Part model, mm, in its own coordinate system. A direction names the side the tool comes from. Give positions to 0.01 mm unless a question says otherwise; leave off trailing zeros. Order: outer loops, then holes, each group sorted by start corner. A loop starts at its lowest first (then second) coordinate and runs counter-clockwise, first axis right, second up. Notation, with made-up numbers: (86.25, 2.5) - (135.25, 2.5) arc R8 cw to (135.25, 17.5) - close; hole circle Ø11 at (57.5, -11.75). An arc over 180 degrees is marked (long way). One line per item, written item: value.
```python
from build123d import *

# Parameters (mm, degrees)
L_BRACKET_BODY_DEPTH          = 47.5
UPRIGHT_ROUND_TOP_DEPTH       = 40
HUB_BOSS_40_SKETCH_R          = 20
HUB_BOSS_40_DEPTH             = 8
BEARING_BORE_30_SKETCH_R      = 15
BEARING_BORE_30_DEPTH         = 65
CLAMP_BORE_40_WITH_SLOT_DEPTH = 65
CLAMP_SCREW_HOLE_10_SKETCH_R  = 5
CLAMP_SCREW_HOLE_10_DEPTH     = 253.833937595


with BuildPart() as part:
    # L-Bracket Profile Sketch → L-Bracket Body (new, symmetric)
    with BuildSketch(Plane.XY):
        with BuildLine():
            Line((0, 0), (150, 0))
            Line((150, 0), (150, 20))
            Line((150, 20), (75, 40))
            Line((75, 40), (55, 40))
            ThreePointArc((55, 40), (44.393398282, 44.393398282), (40, 55))
            Line((40, 55), (40, 132.5))
            Line((40, 132.5), (0, 132.5))
            Line((0, 132.5), (0, 0))
        make_face()
    extrude(amount=L_BRACKET_BODY_DEPTH, both=True)

    # Upright Round Top Sketch → Upright Round Top (add)
    with BuildSketch(Plane.ZY):
        with BuildLine():
            Line((-47.5, 132.5), (47.5, 132.5))
            ThreePointArc((47.5, 132.5), (0, 180), (-47.5, 132.5))
        make_face()
    extrude(amount=-UPRIGHT_ROUND_TOP_DEPTH)

    # Hub Boss Ø40 Sketch → Hub Boss Ø40 (add)
    with BuildSketch(Plane(origin=(40, 0, 0), x_dir=(0, 0, -1), z_dir=(1, 0, 0))):
        with Locations(Location((0, 132.5, 0), (0, 0, 270))):
            Circle(HUB_BOSS_40_SKETCH_R)
    extrude(amount=HUB_BOSS_40_DEPTH)

    # Bearing Bore Ø30 Sketch → Bearing Bore Ø30 (cut)
    with BuildSketch(Plane(origin=(48, 0, 0), x_dir=(0, 0, -1), z_dir=(1, 0, 0))):
        with Locations(Location((0, 132.5, 0), (0, 0, 90))):
            Circle(BEARING_BORE_30_SKETCH_R)
    extrude(amount=-BEARING_BORE_30_DEPTH, mode=Mode.SUBTRACT)

    # Clamp Bore Ø40 Slot Sketch → Clamp Bore Ø40 with Slot (cut)
    with BuildSketch(Plane(origin=(0, 40, 0), x_dir=(1, 0, 0), z_dir=(0, 1, 0))):
        with BuildLine():
            Line((150, 5), (150, -5))
            Line((150, -5), (129.364916731, -5))
            ThreePointArc((129.364916731, -5), (110, -20), (90.635083269, -5))
            Line((90.635083269, -5), (55, -5))
            Line((55, -5), (55, 5))
            Line((55, 5), (90.635083269, 5))
            ThreePointArc((90.635083269, 5), (110, 20), (129.364916731, 5))
            Line((129.364916731, 5), (150, 5))
        make_face()
    extrude(amount=-CLAMP_BORE_40_WITH_SLOT_DEPTH, mode=Mode.SUBTRACT)

    # Clamp Screw Hole Ø10 Sketch → Clamp Screw Hole Ø10 (cut, through all)
    with BuildSketch(Plane.XY.offset(47.5)):
        with Locations((140, 10)):
            Circle(CLAMP_SCREW_HOLE_10_SKETCH_R)
    extrude(amount=-CLAMP_SCREW_HOLE_10_DEPTH, mode=Mode.SUBTRACT)


solid = part.part
```
1) Slice it at C-C on x = 113.5. Write the cut outline in (y, z).
Answer:
outline: (0, -47.5) - (29.73, -47.5) - (29.73, -19.69) - (0, -19.69) - close; (0, 19.69) - (29.73, 19.69) - (29.73, 47.5) - (0, 47.5) - close
2) Slice it at D-D on z = 0. Write the cut outline in (x, y).
Answer:
outline: (0, 0) - (55, 0) - (55, 40) arc R15 cw to (40, 55) - (40, 112.5) - (48, 112.5) - (48, 117.5) - (0, 117.5) - close; (0, 147.5) - (48, 147.5) - (48, 152.5) - (40, 152.5) - (40, 180) - (0, 180) - close
3) Drop flat-ended pins along their axis: P1, Ø12, axis at x = 32.5, z = -3.5, coming from the +Y side; P2, Ø22, axis at x = 67.5, z = -17.5, coming from the +Y side; P3, Ø12, axis at x = 89.5, z = 31.5, coming from the +Y side. Give the stop position or say it passes through.
Answer:
P1: stops at y = 180
P2: stops at y = 40
P3: stops at y = 37.73
4) Slice it at B-B on y = 10. Write the cut outline in (x, z).
Answer:
outline: (0, -47.5) - (135, -47.5) - (135, -5) - (129.36, -5) arc R20 cw to (90.64, -5) - (55, -5) - (55, 5) - (90.64, 5) arc R20 cw to (129.36, 5) - (135, 5) - (135, 47.5) - (0, 47.5) - close; (145, -47.5) - (150, -47.5) - (150, -5) - (145, -5) - close; (145, 5) - (150, 5) - (150, 47.5) - (145, 47.5) - close
5) Slice it at A-A on z = 11. Write the cut outline in (x, y).
Answer:
outline: (0, 0) - (93.3, 0) - (93.3, 35.12) - (75, 40) - (55, 40) arc R15 cw to (40, 55) - (40, 115.8) - (48, 115.8) - (48, 122.3) - (0, 122.3) - close; (0, 142.7) - (48, 142.7) - (48, 149.2) - (40, 149.2) - (40, 178.71) - (0, 178.71) - close; (126.7, 0) - (150, 0) - (150, 20) - (126.7, 26.21) - close; hole circle Ø10 at (140, 10)
6) Which spindle directions (+Z, -Z, +X, -X, +Y, -Y) get a long thin tool onto all of the face, cutting with end or side? Do faces 1 (the face through (65, 40, -26)), 2 (the face through (40, 104, -1)), 3 (the face through (140, 16, 5)), 4 (the face through (110, 14, 20)). Say none if no direction does.
Answer:
face 1: +Z, -Z, +X, +Y
face 2: +X
face 3: +X, +Y, -Y
face 4: +Y, -Y
7) Wall check: line 1 along Z through (x, y) = (30.5, 132.5); line 2 along X through (y, z) = (124, 20). Give the ranges that are in metal, low to high. Write a range as [from, to].
Answer:
line 1: z = [-47.5, -15], [15, 47.5]
line 2: x = [0, 40]
8) Two-plate mould, pull along Z, no slides. Class faces 5 (the face through (55, 20, 0)), 6 (the face through (41, 38, -47.5)), 7 (the face through (48, 130, -15)): pulls with the +Z half, pulls with the -Z half, needs draft (parallel to the pull), parting line crosses it, or undercut.
Answer:
face 5: undercut
face 6: pulls with the -Z half
face 7: needs draft
